from build123d import *

# Parameters (mm, degrees)
BOSS_EXTRUDE1_DEPTH            = 45
SKETCH9_W                      = 2
SKETCH9_H                      = 60
CUT_EXTRUDE1_DEPTH             = 143.049287221
M5_TAPPED_HOLE2_D              = 4.2
F_5_5_5_5_DIAMETER_HOLE1_D     = 5.5
F_5_5_5_5_DIAMETER_HOLE1_DEPTH = 20
F_5_5_5_5_DIAMETER_HOLE1_TIP   = 1.652366702
CHAMFER1_SIZE                  = 1
M5_TAPPED_HOLE3_D              = 4.2
M5_TAPPED_HOLE3_DEPTH          = 14
M5_TAPPED_HOLE3_TIP            = 1.2618073
CUT_EXTRUDE2_REACH             = 144.049


with BuildPart() as part:
    # Sketch1 → Boss-Extrude1 (new body)
    with BuildSketch(Plane.XY):
        Polygon((27, 0), (-27, 0), (-27, 12), (-12, 12), (-12, 132), (12, 132), (12, 12), (27, 12), align=None)
    extrude(amount=BOSS_EXTRUDE1_DEPTH)

    # Sketch9 → Cut-Extrude1 (cut, through all)
    with BuildSketch(Plane.XY.offset(45)):
        with Locations((-11, 102)):
            Rectangle(SKETCH9_W, SKETCH9_H)
        with Locations((11, 102)):
            Rectangle(SKETCH9_W, SKETCH9_H)
    extrude(amount=-CUT_EXTRUDE1_DEPTH, mode=Mode.SUBTRACT)

    # M5 Tapped Hole2 (through all)
    with Locations(Plane(origin=(10, -0.235974088, -1.632115168), x_dir=(0, 0, -1), z_dir=(1, 0, 0))):
        with Locations((-8.632115168, 102.235974088), (-24.632115168, 87.235974088)):
            Hole(M5_TAPPED_HOLE2_D / 2)

    # Ø5.5 (5.5) Diameter Hole1
    with Locations(Plane(origin=(0, 12, 0), x_dir=(-1, 0, 0), z_dir=(0, 1, 0))):
        with Locations((20, 7.5), (20, 37.5), (-20, 37.5), (-20, 7.5)):
            Hole(F_5_5_5_5_DIAMETER_HOLE1_D / 2, depth=F_5_5_5_5_DIAMETER_HOLE1_DEPTH)
            with Locations((0, 0, -(F_5_5_5_5_DIAMETER_HOLE1_DEPTH + F_5_5_5_5_DIAMETER_HOLE1_TIP / 2))):  # 118° drill point
                Cone(0, F_5_5_5_5_DIAMETER_HOLE1_D / 2, F_5_5_5_5_DIAMETER_HOLE1_TIP, mode=Mode.SUBTRACT)

    # Chamfer1
    chamfer1_edges = [part.edges().sort_by_distance(p)[0] for p in [
        (27, 6, 45),
        (-27, 6, 0),
        (-27, 6, 45),
        (27, 6, 0),
    ]]
    chamfer(chamfer1_edges, length=CHAMFER1_SIZE)

    # M5 Tapped Hole3
    with Locations(Plane(origin=(0, 132, 0), x_dir=(-1, 0, 0), z_dir=(0, 1, 0))):
        with Locations((0, 37.5), (0, 7.5)):
            Hole(M5_TAPPED_HOLE3_D / 2, depth=M5_TAPPED_HOLE3_DEPTH)
            with Locations((0, 0, -(M5_TAPPED_HOLE3_DEPTH + M5_TAPPED_HOLE3_TIP / 2))):  # 118° drill point
                Cone(0, M5_TAPPED_HOLE3_D / 2, M5_TAPPED_HOLE3_TIP, mode=Mode.SUBTRACT)

    # Sketch12 → Cut-Extrude2 (cut, up to next)
    with BuildSketch(Plane.XZ, mode=Mode.PRIVATE) as cut_extrude2_sk1:
        with BuildLine():
            Line((-17.25, 37.5), (-17.25, 7.5))
            ThreePointArc((-17.25, 7.5), (-20, 4.75), (-22.75, 7.5))
            Line((-22.75, 7.5), (-22.75, 37.5))
            ThreePointArc((-22.75, 37.5), (-20, 40.25), (-17.25, 37.5))
        make_face()
    cut_extrude2_tool1 = extrude(cut_extrude2_sk1.sketch, amount=-CUT_EXTRUDE2_REACH, mode=Mode.PRIVATE) & part.part
    # Sketch12 → Cut-Extrude2 (cut, up to next)
    with BuildSketch(Plane.XZ, mode=Mode.PRIVATE) as cut_extrude2_sk2:
        with BuildLine():
            Line((22.75, 37.5), (22.75, 7.5))
            ThreePointArc((22.75, 7.5), (20, 4.75), (17.25, 7.5))
            Line((17.25, 7.5), (17.25, 37.5))
            ThreePointArc((17.25, 37.5), (20, 40.25), (22.75, 37.5))
        make_face()
    cut_extrude2_tool2 = extrude(cut_extrude2_sk2.sketch, amount=-CUT_EXTRUDE2_REACH, mode=Mode.PRIVATE) & part.part
    add(cut_extrude2_tool1.solids().sort_by_distance((-20, 0, 22.5))[0], mode=Mode.SUBTRACT)
    add(cut_extrude2_tool2.solids().sort_by_distance((20, 0, 22.5))[0], mode=Mode.SUBTRACT)


solid = part.part
Input: part model. Units: mm. Frame: model coordinates. A direction names the side the tool comes from. Give positions to 0.01 mm unless a question says otherwise; leave off trailing zeros. Order: outer loops, then holes, each group sorted by start corner. A loop starts at its lowest first (then second) coordinate and runs counter-clockwise, first axis right, second up. Notation, with made-up numbers: (36, 51.5) - (55, 51.5) arc R20 ccw to (55, 59.5) - close; hole circle Ø5 at (16, -6). An arc over 180 degrees is marked (long way). Answer as a JSON object with one key per item and string values. Group by question number.
Q1. Cut plane B-B, the plane x = -20. Output: boundary loops of the cut face in (y, z).
Q2. Cut plane C-C, the plane z = 29. Output: boundary loops of the cut face in (x, y), then the cut area to 3 significant figures.
Q3. First-contact query: pin 1 Ø2 at (y, z) = (107.5, 33.5) entering from +X; pin 2 Ø12 at (x, z) = (23, 28.5) entering from +Y; pin 3 Ø22.5 at (y, z) = (38.5, 16) entering from -X. Flat tips, straight axial feed; report the tip coordinate or a pass-through.
Q4. Line query: probe 1 along Z at (x, y) = (0, 124.75); probe 2 along Y at (x, z) = (5.75, 23); probe 3 along X at (y, z) = (8, 39.5). Output: solid intervals per line, ascending.
Q5. Cut plane A-A, the plane y = 102. Output: boundary loops of the cut face in (x, z).
Q6. Cut plane D-D, the plane z = 23. Output: boundary loops of the cut face in (x, y), then the cut area to 3 significant figures.
Q7. Mould query, pull axis X, two halves, no side actions, for faces 5 (the face through (-12, 42, 22)), 6 (the face through (20.06, 5.92, 40.25)), 7 (the face through (27, 6, 22)), 8 (the face through (-0.46, 124.9, 35.45)). Classes: pulls with the +X half, pulls with the -X half, needs draft (parallel to the pull), parting line crosses it, or undercut.
Q8. Set-up query: faces 1 (the face through (10, 102, 23)), 2 (the face through (-0.273, 124.902, 9.582)), 3 (the face through (-19.94, 5.92, 40.25)), 4 (the face through (-10, 102, 23)). Return all of +Z, -Z, +X, -X, +Y, -Y with unobstructed straight access to the full face (end or side cutting, diameter ignored); none if empty.
Results:
{
 "1": {"outline": "(0, 0) - (12, 0) - (12, 4.75) - (0, 4.75) - close; (0, 40.25) - (12, 40.25) - (12, 45) - (0, 45) - close"},
 "2": {"outline": "(-27, 0) - (-22.75, 0) - (-22.75, 12) - (-27, 12) - close; (-17.25, 0) - (17.25, 0) - (17.25, 12) - (12, 12) - (12, 72) - (10, 72) - (10, 132) - (-10, 132) - (-10, 72) - (-12, 72) - (-12, 12) - (-17.25, 12) - close; (22.75, 0) - (27, 0) - (27, 12) - (22.75, 12) - close", "area": "3,160 mm^2"},
 "3": {"pin 1": "x = 10", "pin 2": "y = 12", "pin 3": "x = -12"},
 "4": {"probe 1": "0 to 5.4, 9.6 to 35.4, 39.6 to 45", "probe 2": "0 to 84.9, 89.1 to 132", "probe 3": "-27 to -21.89, -18.11 to 18.11, 21.89 to 27"},
 "5": {"outline": "(-10, 0) - (10, 0) - (10, 4.9) - (-10, 4.9) - close; (-10, 9.1) - (10, 9.1) - (10, 45) - (-10, 45) - close"},
 "6": {"outline": "(-27, 0) - (-22.75, 0) - (-22.75, 12) - (-27, 12) - close; (-17.25, 0) - (17.25, 0) - (17.25, 12) - (12, 12) - (12, 72) - (10, 72) - (10, 84.9) - (-10, 84.9) - (-10, 72) - (-12, 72) - (-12, 12) - (-17.25, 12) - close; (-10, 89.1) - (10, 89.1) - (10, 132) - (-10, 132) - close; (22.75, 0) - (27, 0) - (27, 12) - (22.75, 12) - close", "area": "3,070 mm^2"},
 "7": {"face 5": "pulls with the -X half", "face 6": "undercut", "face 7": "pulls with the +X half", "face 8": "undercut"},
 "8": {"face 1": "+Z, -Z, +X, +Y", "face 2": "+Y", "face 3": "+Y, -Y", "face 4": "+Z, -Z, -X, +Y"}
}
